For this review, take the finished solid that the model builds, in its own axes (mm). A direction names the side the tool comes from. Coordinates: 2 decimals unless noted, no trailing zeros. Loops run counter-clockwise (first coordinate to the right, second up) from the corner with the lowest first, then second, coordinate; pieces in that order, holes last. Notation, with made-up numbers: (68.5, -10) - (86.5, -10) arc R37 ccw to (86.5, 28) - close; hole circle Ø2 at (69.25, -26). An arc over 180 degrees is marked (long way). One line per item, written item: value. Start each with the question number.
1. Take a section at C-C, the plane y = -0.55. State the section outline as (x, z) points.
2. Take a section at B-B, the plane z = -14.5. State the section outline as (x, y) points, and give its area (3 significant figures).
3. For faces 1 (the face through (-38.668, -2.24, 5.077)), 2 (the face through (-37, 0, -6)), 3 (the face through (40, -1, 9)), list the 3-axis set-ups (+Z, -Z, +X, -X, +Y, -Y) from which the entire face can be reached by the end or side of a thin tool; tool diameter is ignored.
4. To check wall thickness, follow line 1 (X direction, y = -1.1, z = 0); line 2 (X direction, y = -2.35, z = 0); line 3 (Z direction, x = -17, y = -0.5). State the ranges of each line that lie inside material, in increasing order. Write a range as from..to.
5. Take a section at A-A, the plane x = 0. State the section outline as (y, z) points.
6. Insertion check: pin 1 (23.5 mm diameter, centred on x = -1.5, z = 17, fed in from -Y). The pin has a flat end and moves straight along its axis. Give the tip position at first contact, or say it passes through.
```python
from build123d import *


with BuildPart() as part:
    # 草图1 → 旋转1 (revolve)
    with BuildSketch(Plane.XY, mode=Mode.PRIVATE) as revolve_1_sk:
        Polygon((-37, 0), (-41, 0), (-41, -1.5), (-43, -1.5), (-43, -3), (-39, -3), (-39, -1.5), (-37, -1.5), align=None)
    revolve(revolve_1_sk.sketch.rotate(Axis((0, 0, 0), (0, 1, 0)), 270), axis=Axis((0, 0, 0), (0, 1, 0)))


solid = part.part
```
Solutions:
1. outline: circle Ø82 at (0, 0); hole circle Ø74 at (0, 0)
2. outline: (-40.48, -3) - (-36.2, -3) - (-36.2, -1.5) - (-34.04, -1.5) - (-34.04, 0) - (-38.35, 0) - (-38.35, -1.5) - (-40.48, -1.5) - close; (34.04, -1.5) - (36.2, -1.5) - (36.2, -3) - (40.48, -3) - (40.48, -1.5) - (38.35, -1.5) - (38.35, 0) - (34.04, 0) - close
2. area: 25.8 mm2
3. face 1: -Y
3. face 2: +Z, -Z, +X, -X, +Y
3. face 3: +Y
4. line 1: -41..-37, 37..41
4. line 2: -43..-39, 39..43
4. line 3: -37.31..-32.86, 32.86..37.31
5. outline: (-3, -43) - (-1.5, -43) - (-1.5, -41) - (0, -41) - (0, -37) - (-1.5, -37) - (-1.5, -39) - (-3, -39) - close; (-3, 39) - (-1.5, 39) - (-1.5, 37) - (0, 37) - (0, 41) - (-1.5, 41) - (-1.5, 43) - (-3, 43) - close
6. pin 1: through
